Design review of the part built by this model. Coordinates are the model's own, in mm. Face numbers are marked on the shaded views. A direction names the side the tool comes from. Give positions to 0.01 mm unless a question says otherwise; leave off trailing zeros. Loops run counter-clockwise (first coordinate to the right, second up) from the corner with the lowest first, then second, coordinate; pieces in that order, holes last.
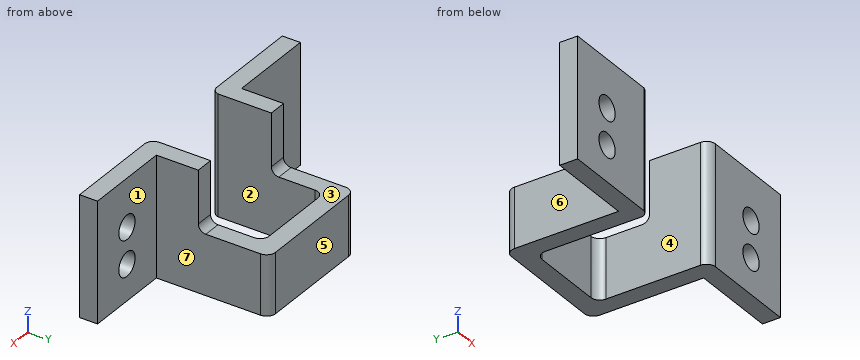
from build123d import *

# Parameters (mm, degrees)
BRACKET_BODY_40MM_DEPTH          = 20
STEPPED_START                    = 28
STEPPED_RELIEF_CUT_28MM_DEPTH    = 28
CORNER_ROUND_CUT_A_R3_DEPTH      = 88.96284726
CORNER_ROUND_CUT_B_R3_DEPTH      = 81.854576235
CORNER_ROUND_CUT_B_R3_DEPTH_BACK = 81.854576235
CORNER_FILL_BOSS_A_6MM_DEPTH     = 6
CORNER_START                     = -6
CORNER_FILL_BOSS_B_6MM_DEPTH     = 6
MOUNTING_HOLES_SKETCH_R          = 4
FLANGE_MOUNTING_HOLES_DEPTH      = 78.77327287


with BuildPart() as part:
    # Bracket Profile Sketch → Bracket Body 40mm (new, symmetric)
    with BuildSketch(Plane.XY):
        with BuildLine():
            Line((30, 0), (65, 0))
            Line((65, 0), (65, 6))
            Line((65, 6), (36, 6))
            Line((36, 6), (36, 40.731710442))
            ThreePointArc((36, 40.731710442), (35.121320344, 42.853030785), (33, 43.731710442))
            Line((33, 43.731710442), (-3, 43.731710442))
            ThreePointArc((-3, 43.731710442), (-5.121320344, 42.853030785), (-6, 40.731710442))
            Line((-6, 40.731710442), (-6, 6))
            Line((-6, 6), (-35, 6))
            Line((-35, 6), (-35, 0))
            Line((-35, 0), (0, 0))
            Line((0, 0), (0, 34.547795072))
            ThreePointArc((0, 34.547795072), (0.878679656, 36.669115416), (3, 37.547795072))
            Line((3, 37.547795072), (27, 37.547795072))
            ThreePointArc((27, 37.547795072), (29.121320344, 36.669115416), (30, 34.547795072))
            Line((30, 34.547795072), (30, 0))
        make_face()
    extrude(amount=BRACKET_BODY_40MM_DEPTH, both=True)

    # Relief Cut Sketch → Stepped Relief Cut 28mm (cut)
    with BuildSketch(Plane.XY.offset(STEPPED_START)):
        with BuildLine():
            Line((33, 43.731710442), (-3, 43.731710442))
            ThreePointArc((-3, 43.731710442), (-5.121320344, 42.853030785), (-6, 40.731710442))
            Line((-6, 40.731710442), (-6, 20))
            Line((-6, 20), (0, 20))
            Line((0, 20), (0, 34.547795072))
            ThreePointArc((0, 34.547795072), (0.878679656, 36.669115416), (3, 37.547795072))
            Line((3, 37.547795072), (27, 37.547795072))
            ThreePointArc((27, 37.547795072), (29.121320344, 36.669115416), (30, 34.547795072))
            Line((30, 34.547795072), (30, 20))
            Line((30, 20), (36, 20))
            Line((36, 20), (36, 40.731710442))
            ThreePointArc((36, 40.731710442), (35.121320344, 42.853030785), (33, 43.731710442))
        make_face()
    extrude(amount=-STEPPED_RELIEF_CUT_28MM_DEPTH, mode=Mode.SUBTRACT)

    # Corner Round Cut A Sketch → Corner Round Cut A R3 (cut, through all)
    with BuildSketch(Plane.XY.offset(20)):
        with BuildLine():
            Line((0, 2.140440117), (0, 0))
            Line((0, 0), (-2.252870035, 0))
            ThreePointArc((-2.252870035, 0), (-0.827692267, 0.755785384), (0, 2.140440117))
        make_face()
    extrude(amount=-CORNER_ROUND_CUT_A_R3_DEPTH, mode=Mode.SUBTRACT)

    # Corner Round Cut B Sketch → Corner Round Cut B R3 (cut, two sides: drawn at the far end of the back side and taken through both)
    with BuildSketch(Plane.XY.offset(-CORNER_ROUND_CUT_B_R3_DEPTH_BACK)):
        with BuildLine():
            Line((30, 0), (30, 3))
            ThreePointArc((30, 3), (30.878679656, 0.878679656), (33, 0))
            Line((33, 0), (30, 0))
        make_face()
    extrude(amount=CORNER_ROUND_CUT_B_R3_DEPTH + CORNER_ROUND_CUT_B_R3_DEPTH_BACK, mode=Mode.SUBTRACT)

    # Corner Fill Boss A Sketch → Corner Fill Boss A 6mm (add)
    with BuildSketch(Plane.ZY.offset(6)):
        with BuildLine():
            Line((0, 20), (0, 22.5))
            ThreePointArc((0, 22.5), (0.732233047, 20.732233047), (2.5, 20))
            Line((2.5, 20), (0, 20))
        make_face()
    extrude(amount=-CORNER_FILL_BOSS_A_6MM_DEPTH)

    # Corner Fill Boss B Sketch → Corner Fill Boss B 6mm (add)
    with BuildSketch(Plane(origin=(36, 0, 0), x_dir=(0, 0, -1), z_dir=(1, 0, 0)).offset(CORNER_START)):
        with BuildLine():
            Line((0, 22.5), (0, 20))
            Line((0, 20), (-2.5, 20))
            ThreePointArc((-2.5, 20), (-0.732233047, 20.732233047), (0, 22.5))
        make_face()
    extrude(amount=CORNER_FILL_BOSS_B_6MM_DEPTH)

    # Mounting Holes Sketch → Flange Mounting Holes (cut, through all)
    with BuildSketch(Plane(origin=(0, 6, 0), x_dir=(1, 0, 0), z_dir=(0, 1, 0))):
        with Locations(Location((50.5, -4, 0), (0, 0, 180))):
            Circle(MOUNTING_HOLES_SKETCH_R)
        with Locations(Location((50.5, 8, 0), (0, 0, 180))):
            Circle(MOUNTING_HOLES_SKETCH_R)
        with Locations((-20.5, -4)):
            Circle(MOUNTING_HOLES_SKETCH_R)
        with Locations((-20.5, 8)):
            Circle(MOUNTING_HOLES_SKETCH_R)
    extrude(amount=-FLANGE_MOUNTING_HOLES_DEPTH, mode=Mode.SUBTRACT)


solid = part.part
Q1. Take a section at A-A (z = -8). Give the boundary of the cut face in (x, y).
Results:
outline: (-35, 0) - (-24.5, 0) - (-24.5, 6) - (-35, 6) - close; (-16.5, 0) - (-2.25, 0) arc R3 ccw to (0, 2.14) - (0, 34.55) arc R3 cw to (3, 37.55) - (27, 37.55) arc R3 cw to (30, 34.55) - (30, 3) arc R3 ccw to (33, 0) - (46.5, 0) - (46.5, 6) - (36, 6) - (36, 40.73) arc R3 ccw to (33, 43.73) - (-3, 43.73) arc R3 ccw to (-6, 40.73) - (-6, 6) - (-16.5, 6) - close; (54.5, 0) - (65, 0) - (65, 6) - (54.5, 6) - close
Q2. Tool access review of the marked faces 1, 2 and 3: name each direction out of +Z, -Z, +X, -X, +Y, -Y from which nothing blocks a thin tool from reaching the whole face with its end or side.
Results:
face 1: +Z, -Z, +X, +Y
face 2: +Z, -Z, -Y
face 3: +Z, +X, -X, +Y
Q3. Take a section at C-C (x = 50.5). Give the boundary of the cut face in (y, z), plus the area to 3 significant figures.
Results:
outline: (0, -20) - (6, -20) - (6, -12) - (0, -12) - close; (0, -4) - (6, -4) - (6, 0) - (0, 0) - close; (0, 8) - (6, 8) - (6, 20) - (0, 20) - close
area: 144 mm2
Q4. Insertion check: pin 1 (1.8 mm diameter, centred on x = 32.5, z = 11, fed in from +Y); pin 2 (9.5 mm diameter, centred on y = 26, z = 9, fed in from +X); pin 3 (8.5 mm diameter, centred on x = -26, z = -2.5, fed in from +Y); pin 4 (5 mm diameter, centred on x = 7, z = -2, fed in from -Y). Each pin has a flat end and moves straight along its axis. Give the tip position at first contact, or say it passes through.
Results:
pin 1: stops at y = 20
pin 2: passes through
pin 3: stops at y = 6
pin 4: stops at y = 37.55
Q5. Take a section at B-B (y = 5). Give the boundary of the cut face in (x, z), plus the area to 3 significant figures.
Results:
outline: (-35, -20) - (0, -20) - (0, 20) - (-35, 20) - close; (30, -20) - (65, -20) - (65, 20) - (30, 20) - close; hole circle Ø8 at (-20.5, -8); hole circle Ø8 at (-20.5, 4); hole circle Ø8 at (50.5, -8); hole circle Ø8 at (50.5, 4)
area: 2,600 mm2
Q6. Wall thickness on line 1 (Z direction, x = -20.5, y = 3); line 2 (X direction, y = 15, z = -8); line 3 (Y direction, x = 24.5, z = -7): over which ranges is each line inside the solid? List them lowest first.
Results:
line 1: z = -20 to -12, -4 to 0, 8 to 20
line 2: x = -6 to 0, 30 to 36
line 3: y = 37.55 to 43.73
Q7. Take a section at D-D (y = 28). Give the boundary of the cut face in (x, z).
Results:
outline: (-6, -20) - (0, -20) - (0, 0) - (-6, 0) - close; (30, -20) - (36, -20) - (36, 0) - (30, 0) - close
Q8. Draft analysis for pull direction X (two halves, no side actions). For the marked faces 4, 5, 6 and 7, state which applies: pulls with the +X half, pulls with the -X half, needs draft (parallel to the pull), parting line crosses it, or undercut.
Results:
face 4: undercut
face 5: needs draft
face 6: pulls with the -X half
face 7: pulls with the +X half
